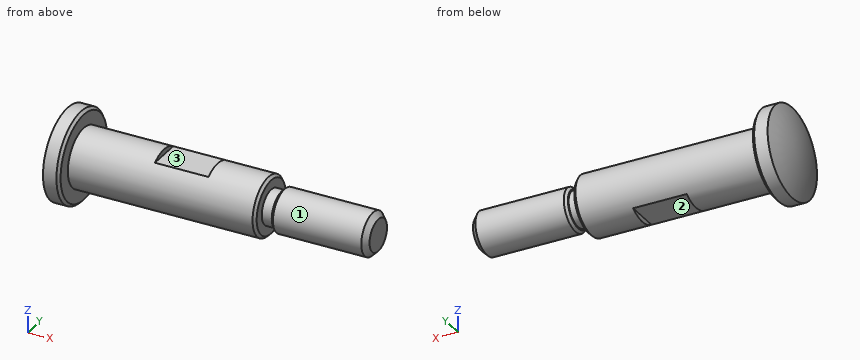
```python
from build123d import *

# Parameters (mm, degrees)
SKETCH2_W          = 10
SKETCH2_H          = 1
CUT_EXTRUDE2_DEPTH = 5
CHAMFER1_SIZE      = 0.5
SKETCH3_W          = 2
SKETCH3_H          = 0.75
CHAMFER2_SIZE      = 0.5


with BuildPart() as part:
    # Sketch1 → Revolve1 (revolve)
    with BuildSketch(Plane.XY, mode=Mode.PRIVATE) as revolve1_sk:
        with BuildLine():
            Line((59.5, 3), (58.5, 4))
            Line((58.5, 4), (39.5, 4))
            Line((39.5, 4), (39.5, 5.5))
            Line((39.5, 5.5), (4.5, 5.5))
            Line((4.5, 5.5), (4.5, 8.5))
            Line((4.5, 8.5), (1.489364109, 8.5))
            ThreePointArc((1.489364109, 8.5), (0.375155866, 4.314748123), (0, 0))
            Line((0, 0), (59.5, 0))
            Line((59.5, 0), (59.5, 3))
        make_face()
    revolve(revolve1_sk.sketch.rotate(Axis((0, 0, 0), (1, 0, 0)), 90), axis=Axis((0, 0, 0), (1, 0, 0)))

    # Sketch2 → Cut-Extrude2 (cut, symmetric)
    with BuildSketch(Plane(origin=(0, 0, 0), x_dir=(1, 0, 0), z_dir=(0, 1, 0))):
        with Locations((24.5, 5)):
            Rectangle(SKETCH2_W, SKETCH2_H)
    cut_extrude2 = extrude(amount=CUT_EXTRUDE2_DEPTH, both=True, mode=Mode.SUBTRACT)

    # Mirror1: Cut-Extrude2 across plane
    add(cut_extrude2.mirror(Plane.XY), mode=Mode.SUBTRACT)

    # Chamfer1
    chamfer1_edges = [part.edges().sort_by_distance(p)[0] for p in [
        (4.5, 0, -8.5),
        (39.5, 0, -5.5),
    ]]
    chamfer(chamfer1_edges, length=CHAMFER1_SIZE)

    # Sketch3 → Cut-Revolve1 (revolve, cut)
    with BuildSketch(Plane(origin=(0, 0, 0), x_dir=(1, 0, 0), z_dir=(0, 1, 0)), mode=Mode.PRIVATE) as cut_revolve1_sk:
        with Locations((40.5, 3.625)):
            Rectangle(SKETCH3_W, SKETCH3_H)
    revolve(cut_revolve1_sk.sketch.rotate(Axis((58.5, 0, 0), (-1, 0, 0)), 270), axis=Axis((58.5, 0, 0), (-1, 0, 0)), mode=Mode.SUBTRACT)

    # Chamfer2
    chamfer2_edges = [part.edges().sort_by_distance(p)[0] for p in [
        (41.5, 0, -4),
    ]]
    chamfer(chamfer2_edges, length=CHAMFER2_SIZE)


solid = part.part
```
The model under review builds one solid part; all positions refer to its coordinate system, in mm. Face numbers are marked on the shaded views. Round coordinates to 2 decimals unless told otherwise and drop trailing zeros. Loops run counter-clockwise (first coordinate to the right, second up) from the corner with the lowest first, then second, coordinate; pieces in that order, holes last. Notation, with made-up numbers: (58, 1.5) - (101, 1.5) arc R12 ccw to (101, 12.5) - close; hole circle Ø11 at (10.5, -22.5). An arc over 180 degrees is marked (long way). Use a Markdown table: item, result. Add a question column.
Q1. Add section C-C (x = 54). State the section outline as (y, z) points, plus the area to 3 significant figures.
Q2. The part is to be moulded in two halves that separate along X. For the marked faces 1, 2 and 3, say which applies: pulls with the +X half, pulls with the -X half, needs draft (parallel to the pull), parting line crosses it, or undercut.
Q3. Insertion check: pin 1 Ø8 at (y, z) = (2, -2.5) entering from +X; pin 2 Ø1 at (x, z) = (25, -4.5) entering from +Y; pin 3 Ø5 at (x, z) = (9.5, 4) entering from -Y; pin 4 Ø1.1 at (y, z) = (0.5, -5) entering from -X. Each pin has a flat end and moves straight along its axis. Give the tip position at first contact, or say it passes through.
Q4. Add section A-A (z = 0). State the section outline as (x, y) points, plus the area to 3 significant figures.
Q5. For probe 1 along X at (y, z) = (0.5, 4.75); probe 2 along Y at (x, z) = (21, -0.25); probe 3 along Z at (x, y) = (24.5, -4.5), list the stretches that pass through material, from the lowest coordinate up.
Worked answers:
| question | item | result |
|---|---|---|
| 1 | outline | circle Ø8 at (0, 0) |
| 1 | area | 50.3 mm² |
| 2 | face 1 | needs draft |
| 2 | face 2 | undercut |
| 2 | face 3 | undercut |
| 3 | pin 1 | x = 59.5 |
| 3 | pin 2 | y = 3.77 |
| 3 | pin 3 | y = -5.29 |
| 3 | pin 4 | x = 0.4 |
| 4 | outline | (1.49, -8.5) - (4, -8.5) - (4.5, -8) - (4.5, -5.5) - (39, -5.5) - (39.5, -5) - (39.5, -3.25) - (41.5, -3.25) - (41.5, -3.5) - (42, -4) - (58.5, -4) - (59.5, -3) - (59.5, 3) - (58.5, 4) - (42, 4) - (41.5, 3.5) - (41.5, 3.25) - (39.5, 3.25) - (39.5, 5) - (39, 5.5) - (4.5, 5.5) - (4.5, 8) - (4, 8.5) - (1.49, 8.5) arc R25 ccw to start |
| 4 | area | 608 mm² |
| 5 | probe 1 | 0.46 to 19.5, 29.5 to 39.5 |
| 5 | probe 2 | -5.49 to 5.49 |
| 5 | probe 3 | -3.16 to 3.16 |
